from build123d import *

# Parameters (mm, degrees)
SKETCH1_R           = 28
BOSS_EXTRUDE1_DEPTH = 6
SKETCH2_R           = 18.5
BOSS_EXTRUDE2_DEPTH = 6
SKETCH3_R           = 14.5
CUT_EXTRUDE1_DEPTH  = 6
FILLET2_R           = 2
CHAMFER1_SIZE       = 1
SKETCH4_R           = 3
CUT_EXTRUDE2_DEPTH  = 6
SKETCH5_W           = 48.146036261
SKETCH5_H           = 7.706921361
CUT_EXTRUDE3_DEPTH  = 6


with BuildPart() as part:
    # Sketch1 → Boss-Extrude1 (new body)
    with BuildSketch(Plane(origin=(0, 0, 0), x_dir=(1, 0, 0), z_dir=(0, 1, 0))):
        with Locations(Location((0, 0, 0), (0, 0, 270))):
            Circle(SKETCH1_R)
    extrude(amount=BOSS_EXTRUDE1_DEPTH)

    # Sketch2 → Boss-Extrude2 (add)
    with BuildSketch(Plane(origin=(0, 6, 0), x_dir=(1, 0, 0), z_dir=(0, 1, 0))):
        with Locations(Location((0, 0, 0), (0, 0, 270))):
            Circle(SKETCH2_R)
    extrude(amount=BOSS_EXTRUDE2_DEPTH)

    # Sketch3 → Cut-Extrude1 (cut)
    with BuildSketch(Plane(origin=(0, 12, 0), x_dir=(1, 0, 0), z_dir=(0, 1, 0))):
        with Locations(Location((0, 0, 0), (0, 0, 270))):
            Circle(SKETCH3_R)
    extrude(amount=-CUT_EXTRUDE1_DEPTH, mode=Mode.SUBTRACT)

    # Fillet2
    fillet2_edges = [part.edges().sort_by_distance(p)[0] for p in [
        (0, 6, -14.5),
    ]]
    fillet(fillet2_edges, radius=FILLET2_R)

    # Chamfer1
    chamfer1_edges = [part.edges().sort_by_distance(p)[0] for p in [
        (0, 0, -28),
        (0, 12, -18.5),
    ]]
    chamfer(chamfer1_edges, length=CHAMFER1_SIZE)

    # Sketch4 → Cut-Extrude2 (cut)
    with BuildSketch(Plane(origin=(0, 6, 0), x_dir=(1, 0, 0), z_dir=(0, 1, 0))):
        with Locations(Location((-16.263455967, 16.263455967, 0), (0, 0, 270))):
            Circle(SKETCH4_R)
        with Locations(Location((16.263455967, 16.263455967, 0), (0, 0, 270))):
            Circle(SKETCH4_R)
        with Locations(Location((16.263455967, -16.263455967, 0), (0, 0, 270))):
            Circle(SKETCH4_R)
        with Locations(Location((-16.263455967, -16.263455967, 0), (0, 0, 270))):
            Circle(SKETCH4_R)
    extrude(amount=-CUT_EXTRUDE2_DEPTH, mode=Mode.SUBTRACT)

    # Sketch5 → Cut-Extrude3 (cut)
    with BuildSketch(Plane(origin=(0, 6, 0), x_dir=(1, 0, 0), z_dir=(0, 1, 0))):
        with Locations((2.860896385, 27.85346068)):
            Rectangle(SKETCH5_W, SKETCH5_H)
    extrude(amount=-CUT_EXTRUDE3_DEPTH, mode=Mode.SUBTRACT)


solid = part.part
Geometry: final body of the model. Coordinates: model frame, mm. A direction names the side the tool comes from. Give positions to 0.01 mm unless a question says otherwise; leave off trailing zeros. Write each loop counter-clockwise with the first axis right and the second up, starting at its lowest first coordinate (ties: lowest second). Pieces come first, ordered by that corner, then holes.
(1) First-contact query: P1, Ø3.5, axis at x = 16.26, z = 16.26, coming from the -Y side; P2, Ø6, axis at y = 2, z = 9, coming from the -X side; P3, Ø1.5, axis at y = 10.5, z = -10, coming from the -X side; P4, Ø1, axis at x = 14.5, y = 7.5, coming from the -Z side. Flat tips, straight axial feed; report the tip coordinate or a pass-through.
(2) Ray query, line 1 (X direction, y = 9, z = 0); line 2 (Z direction, x = -18.5, y = 3.75); line 3 (Z direction, x = -15, y = 4.5). Return the intervals inside material, ascending.
(3) Cut plane B-B, the plane z = 0. Return loops of the section in (x, y).
(4) Access query for faces 1 (the flat face through (13, 12, -7)), 2 (the flat face through (0, 6, 19)). Directions: +Z, -Z, +X, -X, +Y, -Y. A direction counts if a zero-diameter tool reaches every point of the face in a straight line with its end or side. Return the directions, or none.
(5) Mould query, pull axis Z, two halves, no side actions, for faces 3 (the flat face through (0, 0, 1)), 4 (the cylindrical face through (-17.412, 3.042, 19.035)), 5 (the conical face through (-1.01, 0.16, 27.14)). Classes: released by +Z, released by -Z, zero draft, split by the parting line, or undercut.
(6) Cut plane C-C, the plane y = 5.25. Return loops of the section in (x, z), then the cut area to 3 significant figures.
(7) Cut plane A-A, the plane x = 0. Return loops of the section in (y, z).
Values follow:
1. P1: passes through
1. P2: stops at x = -27.35
1. P3: stops at x = -16.02
1. P4: stops at z = -12.09
2. line 1: x = -18.5 to -14.5, 14.5 to 18.5
2. line 2: z = -21.02 to -18.26, -14.26 to 14.26, 18.26 to 21.02
2. line 3: z = -23.64 to -18.98, -13.54 to 13.54, 18.98 to 23.64
3. outline: (-28, 1) - (-27, 0) - (27, 0) - (28, 1) - (28, 6) - (18.5, 6) - (18.5, 11) - (17.5, 12) - (14.5, 12) - (14.5, 8) arc R2 cw to (12.5, 6) - (-12.5, 6) arc R2 cw to (-14.5, 8) - (-14.5, 12) - (-17.5, 12) - (-18.5, 11) - (-18.5, 6) - (-28, 6) - close
4. face 1: +Z, -Z, +X, -X, +Y
4. face 2: +Y
5. face 3: zero draft
5. face 4: undercut
5. face 5: split by the parting line
6. outline: (-14.42, -24) - (14.42, -24) arc R28 ccw (long way) to start; hole circle Ø6 at (-16.26, -16.26); hole circle Ø6 at (-16.26, 16.26); hole circle Ø6 at (16.26, -16.26); hole circle Ø6 at (16.26, 16.26)
6. area: 2,270 mm2
7. outline: (0, -24) - (6, -24) - (6, -18.5) - (11, -18.5) - (12, -17.5) - (12, -14.5) - (8, -14.5) arc R2 cw to (6, -12.5) - (6, 12.5) arc R2 cw to (8, 14.5) - (12, 14.5) - (12, 17.5) - (11, 18.5) - (6, 18.5) - (6, 28) - (1, 28) - (0, 27) - close
